```python
from build123d import *

# Parameters (mm, degrees)
CHAMFER1_SIZE = 1


with BuildPart() as part:
    # Sketch1 → Revolve1 (revolve)
    with BuildSketch(Plane.XY, mode=Mode.PRIVATE) as revolve1_sk:
        Polygon((30, -15), (20, -15), (20, -25), (0, -25), (0, -30), (-5, -30), (-5, 0), (30, 0), align=None)
    revolve(revolve1_sk.sketch.rotate(Axis((30, 0, 0), (-1, 0, 0)), 180), axis=Axis((30, 0, 0), (-1, 0, 0)))

    # Chamfer1
    chamfer1_edges = [part.edges().sort_by_distance(p)[0] for p in [
        (30, -15, 0),
        (20, -25, 0),
        (0, -30, 0),
        (-5, -30, 0),
    ]]
    chamfer(chamfer1_edges, length=CHAMFER1_SIZE)


solid = part.part
```
Model file for the job. Use its own axes, mm. A direction names the side the tool comes from. Coordinates: 2 decimals unless noted, no trailing zeros. Write each loop counter-clockwise with the first axis right and the second up, starting at its lowest first coordinate (ties: lowest second). Pieces come first, ordered by that corner, then holes. Notation, with made-up numbers: (4, -14) - (44, -14) arc R19 cw to (44, 18) - close; hole circle Ø8 at (-38.5, -20). An arc over 180 degrees is marked (long way). Use a Markdown table: item, result. Add a question column.
Item 1: Band-saw the part on C-C, the plane x = 10. Write the cut outline in (y, z), and give its area (3 significant figures).
Item 2: Drop flat-ended pins along their axis: pin 1 (8 mm diameter, centred on x = 19, y = -7, fed in from +Z); pin 2 (12 mm diameter, centred on x = 9.5, z = -6, fed in from -Y); pin 3 (10 mm diameter, centred on y = -2.5, z = -20.5, fed in from +X). Give the stop position or say it passes through.
Item 3: Band-saw the part on D-D, the plane x = 27.5. Write the cut outline in (y, z).
Item 4: 3-axis set-ups, long thin cutter, end or side, ignore diameter. For faces 1 (the face through (-5, 0, 0)), 2 (the face through (20, 0, 16)): which of +Z, -Z, +X, -X, +Y, -Y reach the whole face in a straight line?
Item 5: Drill centre lines: line 1 along X through (y, z) = (25.5, 13); line 2 along X through (y, z) = (-5, -20.5); line 3 along Z through (x, y) = (-1, -25.5). Where is each one in solid material? Low to high.
Item 6: Band-saw the part on A-A, the plane z = 0. Write the cut outline in (x, y).
A:
| question | item | result |
|---|---|---|
| 1 | outline | circle Ø50 at (0, 0) |
| 1 | area | 1,960 mm² |
| 2 | pin 1 | stops at z = 24.82 |
| 2 | pin 2 | stops at y = -25 |
| 2 | pin 3 | stops at x = 20 |
| 3 | outline | circle Ø30 at (0, 0) |
| 4 | face 1 | +Z, -Z, -X, +Y, -Y |
| 4 | face 2 | +X |
| 5 | line 1 | x = -5 to 0 |
| 5 | line 2 | x = -5 to 20 |
| 5 | line 3 | z = -15.8 to 15.8 |
| 6 | outline | (-5, -29) - (-4, -30) - (-1, -30) - (0, -29) - (0, -25) - (19, -25) - (20, -24) - (20, -15) - (29, -15) - (30, -14) - (30, 14) - (29, 15) - (20, 15) - (20, 24) - (19, 25) - (0, 25) - (0, 29) - (-1, 30) - (-4, 30) - (-5, 29) - close |
